Can you work these out from the drawing? Everything is in mm from the part's minimum corner. A direction names the side the tool comes from. Round coordinates to 2 decimals unless told otherwise and drop trailing zeros. Order: outer loops, then holes, each group sorted by start corner. A loop starts at its lowest first (then second) coordinate and runs counter-clockwise, first axis right, second up. Notation, with made-up numbers: (-10.5, 31.5) - (41.5, 31.5) arc R11 cw to (41.5, 46.5) - close; hole circle Ø1 at (73.25, 76). An arc over 180 degrees is marked (long way). Write item = value, one per line.
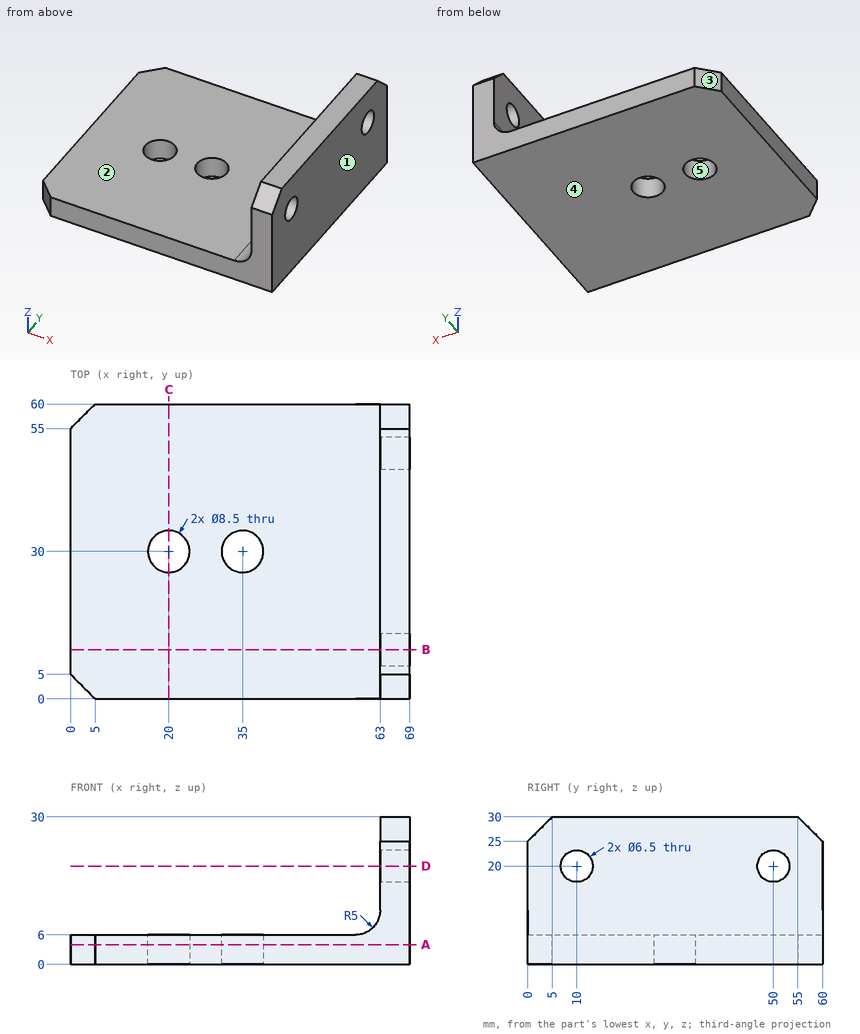
(1) Thinking about a two-plate mould opening in Y: for the marked faces 3, 4 and 5, which applies, +Y half, -Y half, draft (parallel to the pull), parting line (faces both ways), or undercut?
Computed:
face_3 = +Y half
face_4 = draft
face_5 = undercut
(2) If we section it at A-A (z = 4): Write out the boundary of the cut face in (x, y).
Computed:
outline = (0, 5) - (5, 0) - (69, 0) - (69, 60) - (5, 60) - (0, 55) - close; hole circle Ø8.5 at (20, 30); hole circle Ø8.5 at (35, 30)
(3) If we section it at C-C (x = 20): Write out the boundary of the cut face in (y, z).
Computed:
outline = (0, 0) - (25.75, 0) - (25.75, 6) - (0, 6) - close; (34.25, 0) - (60, 0) - (60, 6) - (34.25, 6) - close
(4) On a 3-axis mill with a long thin cutter (end or side, diameter ignored), from which of +Z, -Z, +X, -X, +Y, -Y can I reach the whole of each face in a straight line? I mean the marked faces 1 and 2. Say none if no direction works.
Computed:
face_1 = +Z, -Z, +X, +Y, -Y
face_2 = +Z, -X, +Y, -Y
(5) Will these pins go through, and if not, where does the flat tip stop? P1, Ø5, axis at x = 7, y = 20.5, coming from the +Z side; P2, Ø7.5, axis at y = 10, z = 20, coming from the -X side; P3, Ø10, axis at x = 54.5, z = 22.5, coming from the +Y side.
Computed:
P1 = 6
P2 = 63
P3 = through
(6) If we section it at B-B (y = 10): Write out the boundary of the cut face in (x, z).
Computed:
outline = (0, 0) - (69, 0) - (69, 16.75) - (63, 16.75) - (63, 11) arc R5 cw to (58, 6) - (0, 6) - close; (63, 23.25) - (69, 23.25) - (69, 30) - (63, 30) - close
(7) If we section it at D-D (z = 20): Write out the boundary of the cut face in (x, y).
Computed:
outline = (63, 0) - (69, 0) - (69, 6.75) - (63, 6.75) - close; (63, 13.25) - (69, 13.25) - (69, 46.75) - (63, 46.75) - close; (63, 53.25) - (69, 53.25) - (69, 60) - (63, 60) - close
(8) If I drill on line 1 (Y direction, x = 20, z = 3.95); line 2 (Z direction, x = 67.3, y = 10); line 3 (X direction, y = 29, z = 2.75), over which ranges is the centre line in solid material (lowest first)? Write a range as from..to.
Computed:
line_1 = 0..25.75, 34.25..60
line_2 = 0..16.75, 23.25..30
line_3 = 0..15.87, 24.13..30.87, 39.13..69
